from build123d import *

# Parameters (mm, degrees)
BASE_PLATE_DEPTH      = 25
FRONT_HUB_SKETCH_R    = 27
FRONT_HUB_54_DEPTH    = 10
REAR_START            = 10
REAR_HUB_SKETCH_R     = 27
REAR_HUB_54_DEPTH     = 10
HUB_BORE_SKETCH_R     = 11.5
HUB_BORE_23_DEPTH     = 50
BEARING_BLOCK_DEPTH   = 45
BLOCK_BORE_SKETCH_R   = 17.912737299
BLOCK_BORE_35_8_DEPTH = 45
LUG_TAB_1_DEPTH       = 7
LUG_START             = 7
LUG_TAB_2_DEPTH       = 7
LUG_HOLE_1_SKETCH_R   = 3
LUG_HOLE_1_6_DEPTH    = 7
LUG_START_2           = -7
LUG_HOLE_2_SKETCH_R   = 3
LUG_HOLE_2_6_DEPTH    = 7


with BuildPart() as part:
    # Base Plate Sketch → Base Plate (new body)
    with BuildSketch(Plane.XY):
        with BuildLine():
            Line((-17.1, 54.374534481), (-108.1, 25.756358438))
            ThreePointArc((-108.1, 25.756358438), (-127, 0), (-108.1, -25.756358438))
            Line((-108.1, -25.756358438), (-108.05082408, -25.771771993))
            Line((-108.05082408, -25.771771993), (-20.094170087, -53.340644245))
            ThreePointArc((-20.094170087, -53.340644245), (56.977991401, -1.583823185), (-17.1, 54.374534481))
        make_face()
    extrude(amount=BASE_PLATE_DEPTH)

    # Front Hub Sketch → Front Hub _54 (add)
    with BuildSketch(Plane.XY.offset(25)):
        with Locations(Location((-100, 0, 0), (0, 0, 252.542396876))):
            Circle(FRONT_HUB_SKETCH_R)
    extrude(amount=FRONT_HUB_54_DEPTH)

    # Rear Hub Sketch → Rear Hub _54 (add)
    with BuildSketch(Plane(origin=(0, 0, 0), x_dir=(-1, 0, 0), z_dir=(0, 0, -1)).offset(REAR_START)):
        with Locations((100, 0)):
            Circle(REAR_HUB_SKETCH_R)
    extrude(amount=-REAR_HUB_54_DEPTH)

    # Hub Bore Sketch → Hub Bore _23 (cut)
    with BuildSketch(Plane.XY.offset(35)):
        with Locations((-100, 0)):
            Circle(HUB_BORE_SKETCH_R)
    extrude(amount=-HUB_BORE_23_DEPTH, mode=Mode.SUBTRACT)

    # Bearing Block Sketch → Bearing Block (add)
    with BuildSketch(Plane.XY.offset(25)):
        with BuildLine():
            Line((-40, 25), (10, 25))
            Line((10, 25), (10, -25))
            Line((10, -25), (-40, -25))
            ThreePointArc((-40, -25), (-65, 0), (-40, 25))
        make_face()
    extrude(amount=BEARING_BLOCK_DEPTH)

    # Block Bore Sketch → Block Bore _35.8 (cut)
    with BuildSketch(Plane.XY.offset(70)):
        with Locations((-40, 0)):
            Circle(BLOCK_BORE_SKETCH_R)
    extrude(amount=-BLOCK_BORE_35_8_DEPTH, mode=Mode.SUBTRACT)

    # Lug Tab 1 Sketch → Lug Tab 1 (add)
    with BuildSketch(Plane.XZ.offset(25)):
        with BuildLine():
            Line((5, 25), (5, 55))
            ThreePointArc((5, 55), (-1, 61), (-7, 55))
            Line((-7, 55), (-7, 25))
            Line((-7, 25), (5, 25))
        make_face()
    extrude(amount=LUG_TAB_1_DEPTH)

    # Lug Tab 2 Sketch → Lug Tab 2 (add)
    with BuildSketch(Plane(origin=(0, 25, 0), x_dir=(1, 0, 0), z_dir=(0, 1, 0)).offset(LUG_START)):
        with BuildLine():
            Line((5, -25), (5, -55))
            ThreePointArc((5, -55), (-1, -61), (-7, -55))
            Line((-7, -55), (-7, -25))
            Line((-7, -25), (5, -25))
        make_face()
    extrude(amount=-LUG_TAB_2_DEPTH)

    # Lug Hole 1 Sketch → Lug Hole 1 _6 (cut)
    with BuildSketch(Plane.XZ.offset(32)):
        with Locations(Location((-1, 55, 0), (0, 0, 270))):
            Circle(LUG_HOLE_1_SKETCH_R)
    extrude(amount=-LUG_HOLE_1_6_DEPTH, mode=Mode.SUBTRACT)

    # Lug Hole 2 Sketch → Lug Hole 2 _6 (cut)
    with BuildSketch(Plane(origin=(0, 32, 0), x_dir=(1, 0, 0), z_dir=(0, 1, 0)).offset(LUG_START_2)):
        with Locations(Location((-1, -55, 0), (0, 0, 90))):
            Circle(LUG_HOLE_2_SKETCH_R)
    extrude(amount=LUG_HOLE_2_6_DEPTH, mode=Mode.SUBTRACT)


solid = part.part
Check sheet for the modelled part. Datum: model origin and axes. Units: mm. A direction names the side the tool comes from. Coordinates: 2 decimals unless noted, no trailing zeros. Write each loop counter-clockwise with the first axis right and the second up, starting at its lowest first coordinate (ties: lowest second). Pieces come first, ordered by that corner, then holes.
Item 1: Mould release check, pull along Y, two halves, no side actions. Record for faces 1 (the face through (-1, 32, 43)), 2 (the face through (-57.895, 0.788, 47.815)), 3 (the face through (56.916, -3.101, 12.325)): released by +Y, released by -Y, zero draft, split by the parting line, or undercut.
Numbers:
face 1: released by +Y
face 2: undercut
face 3: split by the parting line
Item 2: Cross-section at A-A on z = 30. Record the boundary of the cut face in (x, y), then the cut area to 3 significant figures.
Numbers:
outline: circle Ø54 at (-100, 0); (-40, -25) - (-7, -25) - (-7, -32) - (5, -32) - (5, -25) - (10, -25) - (10, 25) - (5, 25) - (5, 32) - (-7, 32) - (-7, 25) - (-40, 25) arc R25 ccw to start; hole circle Ø23 at (-100, 0); hole circle Ø35.83 at (-40, 0)
area: 4,520 mm2
Item 3: Cross-section at C-C on x = -100. Record the boundary of the cut face in (y, z), then the cut area to 3 significant figures.
Numbers:
outline: (-28.3, 0) - (-27, 0) - (-27, -10) - (-11.5, -10) - (-11.5, 35) - (-27, 35) - (-27, 25) - (-28.3, 25) - close; (11.5, -10) - (27, -10) - (27, 0) - (28.3, 0) - (28.3, 25) - (27, 25) - (27, 35) - (11.5, 35) - close
area: 1,460 mm2
Item 4: Depth check by flat-ended pin: pin 1 Ø8 at (x, z) = (-12.5, 24) entering from -Y; pin 2 Ø3.5 at (y, z) = (-29.5, 45.5) entering from +X; pin 3 Ø9.5 at (x, z) = (-0.5, 36) entering from +Y. Enter the tip coordinate at first touch or a pass-through.
Numbers:
pin 1: stops at y = -56.36
pin 2: stops at x = 5
pin 3: stops at y = 32
Item 5: Scan lines: probe 1 along Y at (x, z) = (-40, 53); probe 2 along X at (y, z) = (-30, 55); probe 3 along Z at (x, y) = (-6.5, 8). Record each from-to range of solid material in increasing order.
Numbers:
probe 1: y = -25 to -17.91, 17.91 to 25
probe 2: x = -7 to -4, 2 to 5
probe 3: z = 0 to 70
Item 6: Cross-section at B-B on y = 0. Record the boundary of the cut face in (x, z).
Numbers:
outline: (-127, -10) - (-111.5, -10) - (-111.5, 35) - (-127, 35) - close; (-88.5, -10) - (-73, -10) - (-73, 0) - (57, 0) - (57, 25) - (10, 25) - (10, 70) - (-22.09, 70) - (-22.09, 25) - (-57.91, 25) - (-57.91, 70) - (-65, 70) - (-65, 25) - (-73, 25) - (-73, 35) - (-88.5, 35) - close
Item 7: Cross-section at D-D on z = 5.5. Record the boundary of the cut face in (x, y).
Numbers:
outline: (-108.1, -25.76) - (-20.09, -53.34) arc R57 ccw (long way) to (-17.1, 54.37) - (-108.1, 25.76) arc R27 ccw to start; hole circle Ø23 at (-100, 0)
Item 8: Access from +Z, -Z, +X, -X, +Y, -Y to the whole of each face (thin tool, end or side, straight path). Record for faces 4 (the face through (-1, 25, 55)), 5 (the face through (-111, 4, 35)), 6 (the face through (-20, -25, 47)).
Numbers:
face 4: +Y
face 5: +Z, -X, +Y, -Y
face 6: +Z, -Y
